Part model, mm, in its own coordinate system. A direction names the side the tool comes from. Coordinates: 2 decimals unless noted, no trailing zeros. Write each loop counter-clockwise with the first axis right and the second up, starting at its lowest first coordinate (ties: lowest second). Pieces come first, ordered by that corner, then holes. Notation, with made-up numbers: (73.25, 17.25) - (84.25, 17.25) arc R20 cw to (84.25, 51.25) - close; hole circle Ø8 at (-7.75, 15). An arc over 180 degrees is marked (long way). Use a Markdown table: item, result.
```python
from build123d import *

# Parameters (mm, degrees)
BASE_BLOCK_SKETCH_W       = 175
BASE_BLOCK_SKETCH_H       = 82
BASE_BLOCK_DEPTH          = 17
SIDE_WALL_DEPTH           = 50
STEP_PAD_SKETCH_W         = 17
STEP_PAD_SKETCH_H         = 82
STEP_PAD_DEPTH            = 3
RAISED_BLOCK_DEPTH        = 17
LUG_BOSS_DEPTH            = 82
LUG_PROFILE_CUT_DEPTH     = 82
KNUCKLE_SLOT_1_DEPTH      = 15
KNUCKLE_START             = -15
KNUCKLE_SLOT_2_DEPTH      = 15
KNUCKLE_RING_2_DEPTH      = 15
KNUCKLE_START_2           = 15
KNUCKLE_RING_1_DEPTH      = 15
CURVED_BRACKET_DEPTH      = 40
BRACKET_TRIM_CUT_SKETCH_R = 10
BRACKET_TRIM_CUT_DEPTH    = 40


with BuildPart() as part:
    # Base Block Sketch → Base Block (new body)
    with BuildSketch(Plane.XY):
        with Locations((87.5, 41)):
            Rectangle(BASE_BLOCK_SKETCH_W, BASE_BLOCK_SKETCH_H)
    extrude(amount=BASE_BLOCK_DEPTH)

    # Side Wall Sketch → Side Wall (add)
    with BuildSketch(Plane.XY.offset(17)):
        with BuildLine():
            Line((175, 82), (175, 0))
            Line((175, 0), (139, 0))
            ThreePointArc((139, 0), (136.878679656, 0.878679656), (136, 3))
            Line((136, 3), (136, 79))
            ThreePointArc((136, 79), (136.878679656, 81.121320344), (139, 82))
            Line((139, 82), (175, 82))
        make_face()
    extrude(amount=SIDE_WALL_DEPTH)

    # Step Pad Sketch → Step Pad (add)
    with BuildSketch(Plane.ZY):
        with Locations((8.5, 41)):
            Rectangle(STEP_PAD_SKETCH_W, STEP_PAD_SKETCH_H)
    extrude(amount=STEP_PAD_DEPTH)

    # Raised Block Sketch → Raised Block (add)
    with BuildSketch(Plane.XY.offset(17)):
        with BuildLine():
            Line((-3, 82), (-3, 0))
            ThreePointArc((-3, 0), (-5.121320344, 0.878679656), (-6, 3))
            Line((-6, 3), (-6, 79))
            ThreePointArc((-6, 79), (-5.121320344, 81.121320344), (-3, 82))
        make_face()
    extrude(amount=-RAISED_BLOCK_DEPTH)

    # Lug Boss Sketch → Lug Boss (add)
    with BuildSketch(Plane.XZ):
        with BuildLine():
            ThreePointArc((75, 17), (40, 52), (5, 17))
            Line((5, 17), (75, 17))
        make_face()
    extrude(amount=-LUG_BOSS_DEPTH)

    # Lug Profile Cut Sketch → Lug Profile Cut (cut)
    with BuildSketch(Plane.XZ):
        with BuildLine():
            Line((30, 0), (50, 0))
            Line((50, 0), (50, 17))
            ThreePointArc((50, 17), (40, 27), (30, 17))
            Line((30, 17), (30, 0))
        make_face()
    extrude(amount=-LUG_PROFILE_CUT_DEPTH, mode=Mode.SUBTRACT)

    # Knuckle Slot 1 Sketch → Knuckle Slot 1 (cut)
    with BuildSketch(Plane.XZ):
        with BuildLine():
            Line((5, 17), (30, 17))
            ThreePointArc((30, 17), (40, 27), (50, 17))
            Line((50, 17), (75, 17))
            ThreePointArc((75, 17), (40, 52), (5, 17))
        make_face()
    extrude(amount=-KNUCKLE_SLOT_1_DEPTH, mode=Mode.SUBTRACT)

    # Knuckle Slot 2 Sketch → Knuckle Slot 2 (cut)
    with BuildSketch(Plane(origin=(0, 82, 0), x_dir=(1, 0, 0), z_dir=(0, 1, 0)).offset(KNUCKLE_START)):
        with BuildLine():
            Line((30, -17), (5, -17))
            ThreePointArc((5, -17), (40, -52), (75, -17))
            Line((75, -17), (50, -17))
            ThreePointArc((50, -17), (40, -27), (30, -17))
        make_face()
    extrude(amount=KNUCKLE_SLOT_2_DEPTH, mode=Mode.SUBTRACT)

    # Knuckle Ring 2 Sketch → Knuckle Ring 2 (add)
    with BuildSketch(Plane(origin=(0, 67, 0), x_dir=(1, 0, 0), z_dir=(0, 1, 0))):
        with BuildLine():
            Line((24, -17), (30, -17))
            ThreePointArc((30, -17), (40, -27), (50, -17))
            Line((50, -17), (56, -17))
            ThreePointArc((56, -17), (40, -33), (24, -17))
        make_face()
    extrude(amount=KNUCKLE_RING_2_DEPTH)

    # Knuckle Ring 1 Sketch → Knuckle Ring 1 (add)
    with BuildSketch(Plane.XZ.offset(-15).offset(KNUCKLE_START_2)):
        with BuildLine():
            Line((24, 17), (30, 17))
            ThreePointArc((30, 17), (40, 27), (50, 17))
            Line((50, 17), (56, 17))
            ThreePointArc((56, 17), (40, 33), (24, 17))
        make_face()
    extrude(amount=-KNUCKLE_RING_1_DEPTH)

    # Curved Bracket Sketch → Curved Bracket (add)
    with BuildSketch(Plane.XY.offset(17)):
        with BuildLine():
            Line((118, 0), (139, 0))
            ThreePointArc((139, 0), (136.878679656, 0.878679656), (136, 3))
            Line((136, 3), (136, 36))
            Line((136, 36), (118, 36))
            ThreePointArc((118, 36), (100, 18), (118, 0))
        make_face()
        with BuildLine():
            Line((118, 82), (139, 82))
            ThreePointArc((139, 82), (136.878679656, 81.121320344), (136, 79))
            Line((136, 79), (136, 46))
            Line((136, 46), (118, 46))
            ThreePointArc((118, 46), (100, 64), (118, 82))
        make_face()
    extrude(amount=CURVED_BRACKET_DEPTH)

    # Bracket Trim Cut Sketch → Bracket Trim Cut (cut)
    with BuildSketch(Plane.XY.offset(57)):
        with Locations((118, 64)):
            Circle(BRACKET_TRIM_CUT_SKETCH_R)
        with Locations((118, 18)):
            Circle(BRACKET_TRIM_CUT_SKETCH_R)
    extrude(amount=-BRACKET_TRIM_CUT_DEPTH, mode=Mode.SUBTRACT)


solid = part.part
```
Item 1: Which spindle directions (+Z, -Z, +X, -X, +Y, -Y) get a long thin tool onto all of the face, cutting with end or side? Do faces 1 (the face through (40, 67, 34)), 2 (the face through (100, 64, 37)), 3 (the face through (40, 7, 33)). Say none if no direction does.
From the geometry:
| item | result |
|---|---|
| face 1 | +Z, +Y |
| face 2 | +Z |
| face 3 | +Z, -Y |
Item 2: Band-saw the part on A-A, the plane z = 50. Give the cut face in (x, y).
From the geometry:
| item | result |
|---|---|
| outline | (28.34, 15) - (51.66, 15) - (51.66, 67) - (28.34, 67) - close; (118, 0) - (175, 0) - (175, 82) - (118, 82) arc R18 ccw to (118, 46) - (136, 46) - (136, 36) - (118, 36) arc R18 ccw to start; hole circle Ø20 at (118, 18); hole circle Ø20 at (118, 64) |
Item 3: Two-plate mould, pull along Y, no slides. Class faces 4 (the face through (100, 18, 37)), 5 (the face through (40, 15, 35)), 6 (the face through (175, 42, 33)): pulls with the +Y half, pulls with the -Y half, needs draft (parallel to the pull), parting line crosses it, or undercut.
From the geometry:
| item | result |
|---|---|
| face 4 | undercut |
| face 5 | pulls with the -Y half |
| face 6 | needs draft |
Item 4: Band-saw the part on D-D, the plane y = 42.5. Give the cut face in (x, z).
From the geometry:
| item | result |
|---|---|
| outline | (-6, 0) - (30, 0) - (30, 17) arc R10 cw to (50, 17) - (50, 0) - (175, 0) - (175, 67) - (136, 67) - (136, 17) - (75, 17) arc R35 ccw to (5, 17) - (-6, 17) - close |
Item 5: Band-saw the part on B-B, the plane y = 64. Give the cut face in (x, z), then the cut area to 3 significant figures.
From the geometry:
| item | result |
|---|---|
| outline | (-6, 0) - (30, 0) - (30, 17) arc R10 cw to (50, 17) - (50, 0) - (175, 0) - (175, 67) - (136, 67) - (136, 57) - (128, 57) - (128, 17) - (108, 17) - (108, 57) - (100, 57) - (100, 17) - (75, 17) arc R35 ccw to (5, 17) - (-6, 17) - close |
| area | 7,090 mm^2 |
Item 6: Band-saw the part on C-C, the plane x = 40. Give the cut face in (y, z), then the cut area to 3 significant figures.
From the geometry:
| item | result |
|---|---|
| outline | (0, 27) - (82, 27) - (82, 33) - (67, 33) - (67, 52) - (15, 52) - (15, 33) - (0, 33) - close |
| area | 1,480 mm^2 |
Item 7: Drop flat-ended pins along their axis: P1, Ø23, axis at x = 118, y = 64, coming from the +Z side; P2, Ø6, axis at x = 61.5, y = 71.5, coming from the +Z side; P3, Ø10, axis at x = 52.5, z = 44, coming from the -Y side. Give the stop position or say it passes through.
From the geometry:
| item | result |
|---|---|
| P1 | z = 57 |
| P2 | z = 17 |
| P3 | y = 15 |
Item 8: Drill centre lines: probe 1 along Y at (x, z) = (118, 37); probe 2 along X at (y, z) = (52, 5); probe 3 along Y at (x, z) = (114, 40). Where is each one in solid material? Low to high.
From the geometry:
| item | result |
|---|---|
| probe 1 | 0 to 8, 28 to 36, 46 to 54, 74 to 82 |
| probe 2 | -6 to 30, 50 to 175 |
| probe 3 | 0.45 to 8.83, 27.17 to 35.55, 46.45 to 54.83, 73.17 to 81.55 |
